Could you check a few things on this model? Use its own coordinates, in mm. A direction names the side the tool comes from. Round coordinates to 2 decimals unless told otherwise and drop trailing zeros. Write each loop counter-clockwise with the first axis right and the second up, starting at its lowest first coordinate (ties: lowest second). Pieces come first, ordered by that corner, then holes. Notation, with made-up numbers: (16.5, 36) -> (20.5, 36) arc R17 ccw to (20.5, 61) -> close; hole circle Ø3 at (16, -13). An arc over 180 degrees is marked (long way). Answer as CSV lines item,"result". Start each with the question number.
Q1. Imagine slicing it at A-A on z = 23.5. Please give me the cut outline in (x, y).
Q2. Will these pins go through, and if not, where does the flat tip stop? pin 1 Ø5 at (x, z) = (6, 14.5) entering from +Y; pin 2 Ø8 at (x, z) = (-2.5, 9.5) entering from +Y; pin 3 Ø8.5 at (x, z) = (2, 25) entering from -Y.
Q3. Imagine slicing it at C-C on z = 11.5. Please give me the cut outline in (x, y), and give its area (3 significant figures).
Q4. For faces 1 (the flat face through (0, 9.5, 25)), 2 (the flat face through (21, -7, 20)), 3 (the cylindrical face through (-2.799, 21.317, 7.605)), which set-ups out of +Z, -Z, +X, -X, +Y, -Y let a thin tool reach every point of the face, with its end or its side?
Q5. Imagine slicing it at D-D on z = 18.75. Please give me the cut outline in (x, y).
Q6. If we mould it in two halves opening along X, with no side actions, what happens to faces 4 (the flat face through (-9, -4, 29)), 5 (the cylindrical face through (-6.94, -31.24, 10.87)), 6 (the flat face through (8.2, -4.8, 25.2))? For each: pulls with the +X half, pulls with the -X half, needs draft (parallel to the pull), parting line crosses it, or undercut.
Q7. Imagine slicing it at B-B on x = 0. Please give me the cut outline in (y, z).
Q8. If I drill on line 1 (Y direction, x = 0, z = 11); line 2 (Z direction, x = 17, y = -24); line 3 (X direction, y = 2.5, z = 10.5), over which ranges is the centre line in solid material (lowest first)? Write a range as [from, to].
from build123d import *

# Parameters (mm, degrees)
SKETCH_1_R              = 32
EXTRUDE_1_DEPTH         = 20
SKETCH_2_R              = 21
EXTRUDE_2_DEPTH         = 9
HOLE_WIZARD_M48_1_D     = 43
HOLE_WIZARD_M48_1_DEPTH = 15
HOLE_WIZARD_M48_1_TIP   = 12.918503309
CUT_EXTRUDE_1_DEPTH     = 54.749418602
CHAMFER_2_SIZE          = 2
CHAMFER_3_SIZE          = 2
FILLET_1_R              = 0.5


with BuildPart() as part:
    # 草图1 → 凸台-拉伸1 (new body)
    with BuildSketch(Plane.XY):
        Circle(SKETCH_1_R)
    extrude(amount=EXTRUDE_1_DEPTH)

    # 草图2 → 凸台-拉伸2 (add)
    with BuildSketch(Plane.XY.offset(20)):
        Circle(SKETCH_2_R)
    extrude(amount=EXTRUDE_2_DEPTH)

    # M48 螺纹孔1
    with Locations(Plane(origin=(0, 0, 0), x_dir=(-1, 0, 0), z_dir=(0, 0, -1))):
        with Locations((0, 0)):
            Hole(HOLE_WIZARD_M48_1_D / 2, depth=HOLE_WIZARD_M48_1_DEPTH)
            with Locations((0, 0, -(HOLE_WIZARD_M48_1_DEPTH + HOLE_WIZARD_M48_1_TIP / 2))):  # 118° drill point
                Cone(0, HOLE_WIZARD_M48_1_D / 2, HOLE_WIZARD_M48_1_TIP, mode=Mode.SUBTRACT)

    # 草图5 → 切除-拉伸1 (cut, through all)
    with BuildSketch(Plane.XY.offset(29)):
        Polygon((10.969655115, 0), (5.484827557, 9.5), (-5.484827557, 9.5), (-10.969655115, 0), (-5.484827557, -9.5), (5.484827557, -9.5), align=None)
    extrude(amount=-CUT_EXTRUDE_1_DEPTH, mode=Mode.SUBTRACT)

    # 倒角2
    chamfer_2_edges = [part.edges().sort_by_distance(p)[0] for p in [
        (-32, 0, 0),
    ]]
    chamfer(chamfer_2_edges, length=CHAMFER_2_SIZE)

    # 倒角3
    chamfer_3_edges = [part.edges().sort_by_distance(p)[0] for p in [
        (-21, 0, 29),
    ]]
    chamfer(chamfer_3_edges, length=CHAMFER_3_SIZE)

    # 圆角1
    fillet_1_edges = [part.edges().sort_by_distance(p)[0] for p in [
        (-21, 0, 20),
    ]]
    fillet(fillet_1_edges, radius=FILLET_1_R)


solid = part.part
Checks:
1,outline,"circle Ø42 at (0, 0); hole (-10.97, 0) -> (-5.48, -9.5) -> (5.48, -9.5) -> (10.97, 0) -> (5.48, 9.5) -> (-5.48, 9.5) -> close"
2,pin 1,"y = 31.81"
2,pin 2,"y = 32"
2,pin 3,"y = -21"
3,outline,"circle Ø64 at (0, 0); hole circle Ø43 at (0, 0)"
3,area,"1,760 mm^2"
4,face 1,"+Z, -Z"
4,face 2,"+Z"
4,face 3,"-Z"
5,outline,"circle Ø64 at (0, 0); hole circle Ø30.52 at (0, 0)"
6,face 4,"needs draft"
6,face 5,"parting line crosses it"
6,face 6,"undercut"
7,outline,"(-32, 2) -> (-30, 0) -> (-21.5, 0) -> (-21.5, 15) -> (-9.5, 22.21) -> (-9.5, 29) -> (-19, 29) -> (-21, 27) -> (-21, 20.5) arc R0.5 cw to (-21.5, 20) -> (-32, 20) -> close; (9.5, 22.21) -> (21.5, 15) -> (21.5, 0) -> (30, 0) -> (32, 2) -> (32, 20) -> (21.5, 20) arc R0.5 cw to (21, 20.5) -> (21, 27) -> (19, 29) -> (9.5, 29) -> close"
8,line 1,"[-32, -21.5], [21.5, 32]"
8,line 2,"[0, 20]"
8,line 3,"[-31.9, -21.35], [21.35, 31.9]"
